For this review, take the finished solid that the model builds, in its own axes (mm). A direction names the side the tool comes from. Coordinates: 2 decimals unless noted, no trailing zeros. Write each loop counter-clockwise with the first axis right and the second up, starting at its lowest first coordinate (ties: lowest second). Pieces come first, ordered by that corner, then holes. Notation, with made-up numbers: (14.25, -33) -> (67.25, -33) arc R20 cw to (67.25, -10) -> close; hole circle Ø7 at (-1, 70). An arc over 180 degrees is marked (long way). One line per item, written item: value. Start each with the question number.
1) Add section D-D (y = -20.5). State the section outline as (x, z) points.
2) Machinability: for faces 5 (the flat face through (16, -9, -9)), 6 (the flat face through (33, 11, -22)), 7 (the cylindrical face through (25.902, 3.307, 12.055)), 8 (the cylindrical face through (25.9, -12.08, -3.21)), 9 (the flat face through (9, 8.15, 0)), which of the approach directions +Z, -Z, +X, -X, +Y, -Y give a long, thin tool a straight path to every point of the face, cutting with its end or side? Answer none if there is none.
3) Add section A-A (y = 0). State the section outline as (x, z) points.
4) For probe 1 along X at (y, z) = (-19, 2.5); probe 2 along X at (y, z) = (-9, -5); probe 3 along Z at (x, y) = (31.5, -20.5), list the stretches that pass through material, from the lowest coordinate up. Write a range as from..to.
5) Add section B-B (x = 29). State the section outline as (y, z) points.
6) Mouldability with a two-part tool opening along Y and no side actions: class faces 1 (the flat face through (33, -15, -21)), 2 (the cylindrical face through (25.9, -8.82, 8.86)), 3 (the cylindrical face through (25.9, 12.08, 3.21)), 4 (the cylindrical face through (7.888, -3.755, 11.923)) as released by +Y, released by -Y, zero draft, split by the parting line, or undercut.
7) For pin 1 Ø0.5 at (x, y) = (6.5, 7.5) entering from -Z; pin 2 Ø16 at (y, z) = (0, 0) entering from +X; pin 3 Ø0.5 at (x, y) = (13, 7) entering from +Z, all flat-tipped, find the tip position at first contact; note any pin that passes through.
8) Add section C-C (z = 0). State the section outline as (x, y) points, and give its area (3 significant figures).
from build123d import *

# Parameters (mm, degrees)
SHAFT_BORE_PROFILE_W = 5
SHAFT_BORE_PROFILE_H = 2.3
SHAFT_BORE_DEPTH     = 30
VANES_6X_DEPTH       = 14


with BuildPart() as part:
    # Hub Disc Profile → Hub and Back Disc (revolve)
    with BuildSketch(Plane.XY, mode=Mode.PRIVATE) as hub_and_back_disc_sk:
        Polygon((0, 12.5), (0, 7), (19, 7), (19, 37.5), (16, 37.5), (16, 12.5), align=None)
    revolve(hub_and_back_disc_sk.sketch.rotate(Axis((-28, 0, 0), (1, 0, 0)), 90), axis=Axis((-28, 0, 0), (1, 0, 0)))

    # Shaft Bore Profile → Shaft Bore (cut)
    with BuildSketch(Plane.ZY):
        with Locations((0, 7)):
            Rectangle(SHAFT_BORE_PROFILE_W, SHAFT_BORE_PROFILE_H)
    extrude(amount=-SHAFT_BORE_DEPTH, mode=Mode.SUBTRACT)

    # Vane Profiles 6x → Vanes 6x (add)
    with BuildSketch(Plane(origin=(19, 0, 0), x_dir=(0, 0, -1), z_dir=(1, 0, 0))):
        with BuildLine():
            ThreePointArc((-36.970311015, -6.2806133), (-36.580104109, -8.255058047), (-36.084528464, -10.205724156))
            ThreePointArc((-36.084528464, -10.205724156), (-21.847293577, -13.468460533), (-7.696370779, -9.849663793))
            ThreePointArc((-7.696370779, -9.849663793), (-8.875739318, -8.801775478), (-9.913722012, -7.613679523))
            ThreePointArc((-9.913722012, -7.613679523), (-23.613958858, -10.436975539), (-36.970311015, -6.2806133))
        make_face()
        with BuildLine():
            ThreePointArc((-13.045984839, -35.157535175), (-11.140962076, -35.806828455), (-9.203847848, -36.352980411))
            ThreePointArc((-9.203847848, -36.352980411), (0.740382183, -25.654541508), (4.681873674, -11.590084508))
            ThreePointArc((4.681873674, -11.590084508), (3.184691504, -12.087503465), (1.636778877, -12.39237487))
            ThreePointArc((1.636778877, -12.39237487), (-2.768293473, -25.668776024), (-13.045984839, -35.157535175))
        make_face()
        with BuildLine():
            ThreePointArc((23.924326177, -28.876921875), (25.439142033, -27.551770408), (26.880680615, -26.147256255))
            ThreePointArc((26.880680615, -26.147256255), (22.58767576, -12.186080975), (12.378244453, -1.740420715))
            ThreePointArc((12.378244453, -1.740420715), (12.060430821, -3.285727987), (11.550500889, -4.778695347))
            ThreePointArc((11.550500889, -4.778695347), (20.845665384, -15.231800485), (23.924326177, -28.876921875))
        make_face()
        with BuildLine():
            ThreePointArc((-1.636778877, 12.39237487), (2.768293473, 25.668776024), (13.045984839, 35.157535175))
            ThreePointArc((13.045984839, 35.157535175), (11.140962076, 35.806828455), (9.203847848, 36.352980411))
            ThreePointArc((9.203847848, 36.352980411), (-0.740382183, 25.654541508), (-4.681873674, 11.590084508))
            ThreePointArc((-4.681873674, 11.590084508), (-3.184691504, 12.087503465), (-1.636778877, 12.39237487))
        make_face()
        with BuildLine():
            ThreePointArc((-23.924326177, 28.876921875), (-20.845665384, 15.231800485), (-11.550500889, 4.778695347))
            ThreePointArc((-11.550500889, 4.778695347), (-12.060430821, 3.285727987), (-12.378244453, 1.740420715))
            ThreePointArc((-12.378244453, 1.740420715), (-22.58767576, 12.186080975), (-26.880680615, 26.147256255))
            ThreePointArc((-26.880680615, 26.147256255), (-25.439142033, 27.551770408), (-23.924326177, 28.876921875))
        make_face()
        with BuildLine():
            ThreePointArc((36.084528464, 10.205724156), (21.847293577, 13.468460533), (7.696370779, 9.849663793))
            ThreePointArc((7.696370779, 9.849663793), (8.875739318, 8.801775478), (9.913722012, 7.613679523))
            ThreePointArc((9.913722012, 7.613679523), (23.613958858, 10.436975539), (36.970311015, 6.2806133))
            ThreePointArc((36.970311015, 6.2806133), (36.580104109, 8.255058047), (36.084528464, 10.205724156))
        make_face()
    extrude(amount=VANES_6X_DEPTH)


solid = part.part
Numbers:
1. outline: (16, -31.4) -> (19, -31.4) -> (19, -26.01) -> (33, -26.01) -> (33, -22.91) -> (19, -22.91) -> (19, -3.04) -> (33, -3.04) -> (33, 0.15) -> (19, 0.15) -> (19, 31.4) -> (16, 31.4) -> close
2. face 5: -X
2. face 6: +Z, -Z, +X, +Y, -Y
2. face 7: -Z, +X
2. face 8: +X
2. face 9: +X, -X
3. outline: (0, -12.5) -> (16, -12.5) -> (16, -37.5) -> (19, -37.5) -> (19, -7) -> (0, -7) -> close; (0, 7) -> (19, 7) -> (19, 37.5) -> (16, 37.5) -> (16, 12.5) -> (0, 12.5) -> close
4. probe 1: 16..19
4. probe 2: 0..19
4. probe 3: -26.01..-22.91, -3.04..0.15
5. outline: (-36.35, 9.2) arc R31 ccw to (-11.59, -4.68) arc R12.5 cw to (-12.39, -1.64) arc R28 cw to (-35.16, 13.05) arc R37.5 ccw to start; (-28.88, -23.92) arc R37.5 ccw to (-26.15, -26.88) arc R31 ccw to (-1.74, -12.38) arc R12.5 cw to (-4.78, -11.55) arc R28 cw to start; (-10.21, 36.08) arc R31 ccw to (-9.85, 7.7) arc R12.5 cw to (-7.61, 9.91) arc R28 cw to (-6.28, 36.97) arc R37.5 ccw to start; (1.74, 12.38) arc R12.5 cw to (4.78, 11.55) arc R28 cw to (28.88, 23.92) arc R37.5 ccw to (26.15, 26.88) arc R31 ccw to start; (6.28, -36.97) arc R37.5 ccw to (10.21, -36.08) arc R31 ccw to (9.85, -7.7) arc R12.5 cw to (7.61, -9.91) arc R28 cw to start; (11.59, 4.68) arc R12.5 cw to (12.39, 1.64) arc R28 cw to (35.16, -13.05) arc R37.5 ccw to (36.35, -9.2) arc R31 ccw to start
6. face 1: zero draft
6. face 2: released by +Y
6. face 3: undercut
6. face 4: split by the parting line
7. pin 1: z = -10.18
7. pin 2: x = 19
7. pin 3: z = 10.52
8. outline: (0, -12.5) -> (16, -12.5) -> (16, -37.5) -> (19, -37.5) -> (19, -26.91) -> (33, -26.91) -> (33, -20.1) -> (19, -20.1) -> (19, -7) -> (0, -7) -> close; (0, 8.15) -> (19, 8.15) -> (19, 20.1) -> (33, 20.1) -> (33, 26.91) -> (19, 26.91) -> (19, 37.5) -> (16, 37.5) -> (16, 12.5) -> (0, 12.5) -> close
8. area: 528 mm²
